from build123d import *

# Parameters (mm, degrees)
SKETCH_1_W      = 1354
SKETCH_1_H      = 40
EXTRUDE_1_DEPTH = 10
SKETCH_2_W      = 40
SKETCH_2_H      = 89
EXTRUDE_2_DEPTH = 10


with BuildPart() as part:
    # 草图1 → 凸台-拉伸1 (new body)
    with BuildSketch(Plane(origin=(0, 0, 0), x_dir=(1, 0, 0), z_dir=(0, 1, 0))):
        Rectangle(SKETCH_1_W, SKETCH_1_H)
    extrude(amount=EXTRUDE_1_DEPTH)

    # 草图2 → 凸台-拉伸2 (add)
    with BuildSketch(Plane.ZY.offset(677)):
        with Locations((0, 44.5)):
            Rectangle(SKETCH_2_W, SKETCH_2_H)
    extrude_2 = extrude(amount=EXTRUDE_2_DEPTH)

    # 镜向1: 凸台-拉伸2 across plane
    add(extrude_2.mirror(Plane(origin=(0, 0, 0), x_dir=(0, 0, 1), z_dir=(1, 0, 0))))


solid = part.part
The model under review builds one solid part; all positions refer to its coordinate system, in mm. A direction names the side the tool comes from. Give positions to 0.01 mm unless a question says otherwise; leave off trailing zeros. Loops run counter-clockwise (first coordinate to the right, second up) from the corner with the lowest first, then second, coordinate; pieces in that order, holes last. Notation, with made-up numbers: (-9, 26.25) -> (9, 26.25) arc R14 ccw to (9, 49.25) -> close; hole circle Ø10 at (64.5, 48). An arc over 180 degrees is marked (long way). Answer as a JSON object with one key per item and string values. Group by question number.
Q1. Tool access review of faces 4 (the flat face through (-3, 5, 20)), 5 (the flat face through (677, 50, 0)): name each direction out of +Z, -Z, +X, -X, +Y, -Y from which nothing blocks a thin tool from reaching the whole face with its end or side.
Q2. Take a section at C-C (x = 248.5). Write out the cut boundary in (y, z).
Q3. Take a section at A-A (y = 70). Write out the cut boundary in (x, z), plus the area to 3 significant figures.
Q4. Wall thickness on line 1 along X through (y, z) = (39, -4.5); line 2 along Y through (x, z) = (10.5, 3): over which ranges is each line inside the solid? List them lowest first.
Q5. Draft analysis for pull direction X (two halves, no side actions). For faces 1 (the flat face through (-10, 0, 0)), 2 (the flat face through (687, 45, 0)), 3 (the flat face through (-9, 10, 0)), state which applies: pulls with the +X half, pulls with the -X half, needs draft (parallel to the pull), parting line crosses it, or undercut.
Q6. Take a section at B-B (z = -6). Write out the cut boundary in (x, y).
Q7. Insertion check: pin 1 (6 mm diameter, centred on x = -363.5, z = 15.5, fed in from +Y). The pin has a flat end and moves straight along its axis. Give the tip position at first contact, or say it passes through.
Answer below:
{
 "1": {"face 4": "+Z, +X, -X, +Y, -Y", "face 5": "+Z, -Z, +Y"},
 "2": {"outline": "(0, -20) -> (10, -20) -> (10, 20) -> (0, 20) -> close"},
 "3": {"outline": "(-687, -20) -> (-677, -20) -> (-677, 20) -> (-687, 20) -> close; (677, -20) -> (687, -20) -> (687, 20) -> (677, 20) -> close", "area": "800 mm2"},
 "4": {"line 1": "x = -687 to -677, 677 to 687", "line 2": "y = 0 to 10"},
 "5": {"face 1": "needs draft", "face 2": "pulls with the +X half", "face 3": "undercut"},
 "6": {"outline": "(-687, 0) -> (687, 0) -> (687, 89) -> (677, 89) -> (677, 10) -> (-677, 10) -> (-677, 89) -> (-687, 89) -> close"},
 "7": {"pin 1": "stops at y = 10"}
}
